For this review, take the finished solid that the model builds, in its own axes (mm). A direction names the side the tool comes from. Coordinates: 2 decimals unless noted, no trailing zeros. Write each loop counter-clockwise with the first axis right and the second up, starting at its lowest first coordinate (ties: lowest second). Pieces come first, ordered by that corner, then holes.
1) For faces 5 (the face through (-5, 0, 279)), 6 (the face through (-0.867, -3.905, 9.62)), 7 (the face through (0, 0, 0)), list the 3-axis set-ups (+Z, -Z, +X, -X, +Y, -Y) from which the entire face can be reached by the end or side of a thin tool; tool diameter is ignored.
2) To check wall thickness, follow line 1 along X through (y, z) = (-6, 183.5); line 2 along Z through (x, y) = (5.5, -0.25); line 3 along Z through (x, y) = (4.75, 5.75). State the ranges of each line that lie inside material, in increasing order.
3) We need section B-B on z = 109.5. Write out the cut boundary in (x, y), then the cut area to 3 significant figures.
4) We need section A-A on z = 28. Write out the cut boundary in (x, y).
5) Insertion check: P1, Ø8, axis at y = 1.5, z = 216, coming from the +X side; P2, Ø3, axis at x = 0, z = 6, coming from the +Y side; P3, Ø4, axis at y = -5, z = 179.5, coming from the -X side; P4, Ø1.5, axis at x = 4.5, z = 208.5, coming from the +Y side. Each pin has a flat end and moves straight along its axis. Give the tip position at first contact, or say it passes through.
6) Mouldability with a two-part tool opening along Z and no side actions: class faces 1 (the face through (-6, 0, 37)), 2 (the face through (-4.745, 0.209, 276.542)), 3 (the face through (2, 5, 268)), 4 (the face through (-4, -2, 19)) as pulls with the +Z half, pulls with the -Z half, needs draft (parallel to the pull), parting line crosses it, or undercut.
from build123d import *

# Parameters (mm, degrees)
SKETCH_1_R          = 7.5
EXTRUDE_1_DEPTH     = 281
SKETCH_3_W          = 48.87377388
SKETCH_3_H          = 13
SKETCH_4_W          = 35.83639091
SKETCH_4_H          = 82.680612398
SKETCH_8_W          = 33.14878911
SKETCH_8_H          = 39.753572134
CHAMFER_2_SIZE      = 0.5
SKETCH_15_W         = 15.290885205
SKETCH_15_H         = 1.1
CHAMFER_3_SIZE      = 0.5
SKETCH_16_W         = 27.071895425
SKETCH_16_H         = 14.859010271
CUT_EXTRUDE_1_DEPTH = 17


with BuildPart() as part:
    # 草图1 → 凸台-拉伸1 (new body)
    with BuildSketch(Plane.XY):
        Circle(SKETCH_1_R)
    extrude(amount=EXTRUDE_1_DEPTH)

    # 草图3 → 切除-旋转1 (revolve, cut)
    with BuildSketch(Plane(origin=(0, 0, 0), x_dir=(1, 0, 0), z_dir=(0, 1, 0)), mode=Mode.PRIVATE) as cut_revolve_1_sk:
        with Locations((-29.43688694, -274.5)):
            Rectangle(SKETCH_3_W, SKETCH_3_H)
    revolve(cut_revolve_1_sk.sketch.rotate(Axis((0, 0, 281), (0, 0, -1)), 180), axis=Axis((0, 0, 281), (0, 0, -1)), mode=Mode.SUBTRACT)

    # 草图4 → 切除-旋转2 (revolve, cut)
    with BuildSketch(Plane(origin=(0, 0, 0), x_dir=(1, 0, 0), z_dir=(0, 1, 0))):
        with Locations((23.918195455, -13.659693801)):
            Rectangle(SKETCH_4_W, SKETCH_4_H)
    revolve(axis=Axis((0, 0, 281), (0, 0, -1)), mode=Mode.SUBTRACT)

    # 草图8 → 切除-旋转5 (revolve, cut)
    with BuildSketch(Plane(origin=(0, 0, 0), x_dir=(1, 0, 0), z_dir=(0, 1, 0)), mode=Mode.PRIVATE) as cut_revolve_5_sk:
        with Locations((-20.574394555, 0.876786067)):
            Rectangle(SKETCH_8_W, SKETCH_8_H)
    revolve(cut_revolve_5_sk.sketch.rotate(Axis((0, 0, 268), (0, 0, 1)), 180), axis=Axis((0, 0, 268), (0, 0, 1)), mode=Mode.SUBTRACT)

    # 倒角2
    chamfer_2_edges = [part.edges().sort_by_distance(p)[0] for p in [
        (-6, 0, 19),
        (-4, 0, 0),
    ]]
    chamfer(chamfer_2_edges, length=CHAMFER_2_SIZE)

    # 草图15 → 切除-旋转7 (revolve, cut)
    with BuildSketch(Plane(origin=(0, 0, 0), x_dir=(1, 0, 0), z_dir=(0, 1, 0)), mode=Mode.PRIVATE) as cut_revolve_7_sk:
        with Locations((-12.395442603, -276.55)):
            Rectangle(SKETCH_15_W, SKETCH_15_H)
    revolve(cut_revolve_7_sk.sketch.rotate(Axis((0, 0, 281), (0, 0, 1)), 180), axis=Axis((0, 0, 281), (0, 0, 1)), mode=Mode.SUBTRACT)

    # 倒角3
    chamfer_3_edges = [part.edges().sort_by_distance(p)[0] for p in [
        (-5, 0, 281),
    ]]
    chamfer(chamfer_3_edges, length=CHAMFER_3_SIZE)

    # 草图16 → 切除-拉伸1 (cut)
    with BuildSketch(Plane(origin=(0, 0, 0), x_dir=(-1, 0, 0), z_dir=(0, 0, -1))):
        with Locations((-4.49502023, 10.929505136)):
            Rectangle(SKETCH_16_W, SKETCH_16_H)
    extrude(amount=-CUT_EXTRUDE_1_DEPTH, mode=Mode.SUBTRACT)


solid = part.part
Result:
1. face 5: +Z
1. face 6: -Z
1. face 7: -Z, +X, -X, +Y, -Y
2. line 1: x = -4.5 to 4.5
2. line 2: z = 19.01 to 268
2. line 3: z = 55 to 268
3. outline: circle Ø15 at (0, 0)
3. area: 177 mm2
4. outline: circle Ø12 at (0, 0)
5. P1: stops at x = 7.5
5. P2: stops at y = 3.5
5. P3: stops at x = -6.87
5. P4: stops at y = 6.5
6. face 1: needs draft
6. face 2: undercut
6. face 3: pulls with the +Z half
6. face 4: pulls with the -Z half
